Part print with two shaded views. Sizes in mm from the minimum x, y, z corner. Give positions to 0.01 mm unless a question says otherwise; leave off trailing zeros. Write each loop counter-clockwise with the first axis right and the second up, starting at its lowest first coordinate (ties: lowest second). Pieces come first, ordered by that corner, then holes.
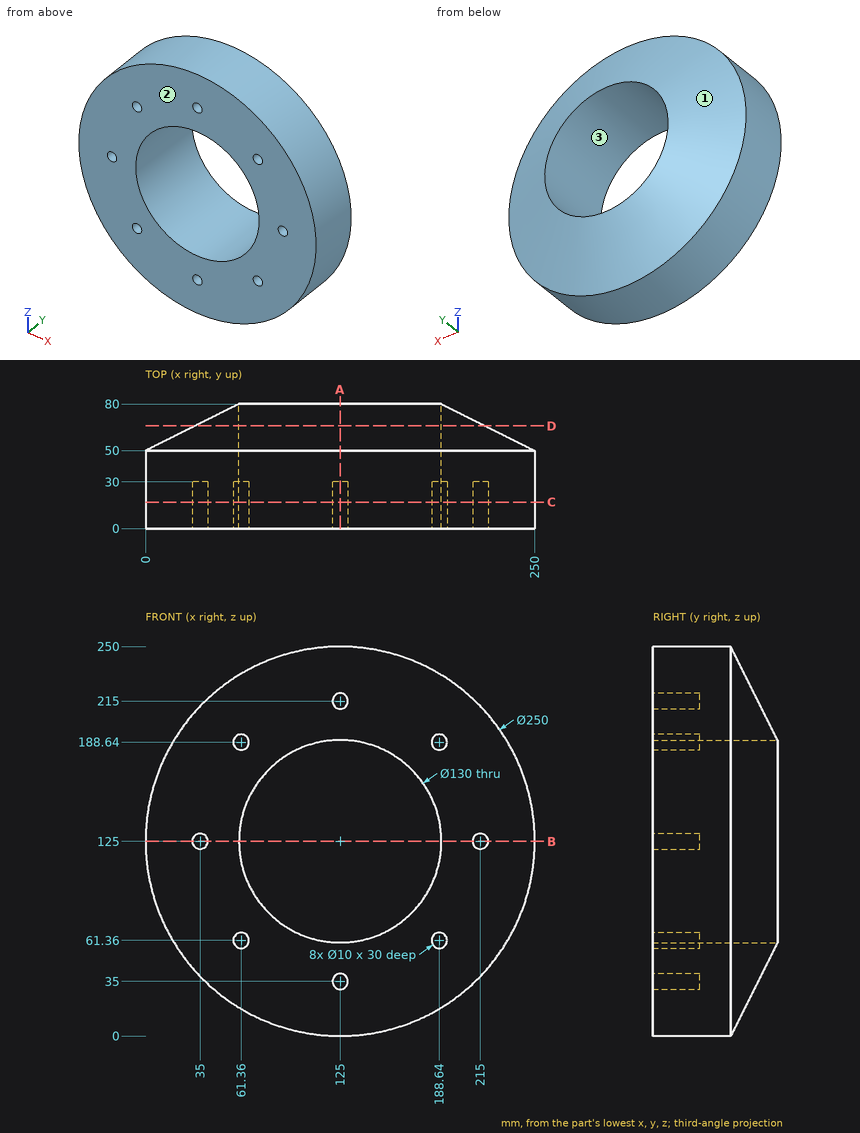
(1) Saw through at C-C, the plane y = 17. Give the number of separate pieces and of enclosed holes in the cut face, plus the area to 3 significant figures.
(2) Saw through at D-D, the plane y = 66. List the corners of the cut face in (x, z), plus the area to 3 significant figures.
(3) Probe line 1 (X direction, y = 18, z = 125); line 2 (X direction, y = 38, z = 125); line 3 (Z direction, x = 162.5, y = 72.5) (1 decimal). List the from-to ranges inside material, lowest first.
(4) Mould opens along X. For the marked faces 1, 2 and 3 say: +X half, -X half, draft (parallel to the pull), parting line (faces both ways), or undercut.
(5) Drop flat-ended pins along their axis: pin 1 (5 mm diameter, centred on x = 70.5, y = 25, fed in from -Z); pin 2 (16 mm diameter, centred on x = 215, z = 125, fed in from -Y); pin 3 (8 mm diameter, centred on x = 125, z = 215, fed in from +Y); pin 4 (16 mm diameter, centred on x = 35, z = 125, fed in from +Y). Give the stop position or say it passes through.
(6) Saw through at A-A, the plane x = 125. List the corners of the cut face in (y, z), plus the area to 3 significant figures.
(7) Saw through at B-B, the plane z = 125. List the corners of the cut face in (x, y), plus the area to 3 significant figures.
Computed values:
1. separate pieces: 1
1. enclosed holes: 9
1. area: 35,200 mm2
2. outline: circle Ø186 at (125, 125); hole circle Ø130 at (125, 125)
2. area: 13,900 mm2
3. line 1: x = 0 to 30, 40 to 60, 190 to 210, 220 to 250
3. line 2: x = 0 to 60, 190 to 250
3. line 3: z = 54.3 to 71.9, 178.1 to 195.7
4. face 1: parting line
4. face 2: draft
4. face 3: undercut
5. pin 1: stops at z = 11.33
5. pin 2: stops at y = 0
5. pin 3: stops at y = 69.5
5. pin 4: stops at y = 71.5
6. outline: (0, 0) - (50, 0) - (80, 60) - (0, 60) - (0, 40) - (30, 40) - (30, 30) - (0, 30) - close; (0, 190) - (80, 190) - (50, 250) - (0, 250) - (0, 220) - (30, 220) - (30, 210) - (0, 210) - close
6. area: 7,200 mm2
7. outline: (0, 0) - (30, 0) - (30, 30) - (40, 30) - (40, 0) - (60, 0) - (60, 80) - (0, 50) - close; (190, 0) - (210, 0) - (210, 30) - (220, 30) - (220, 0) - (250, 0) - (250, 50) - (190, 80) - close
7. area: 7,200 mm2
